```python
from build123d import *


with BuildPart() as part:
    # Sketch1 → Revolve1 (revolve)
    with BuildSketch(Plane.XY, mode=Mode.PRIVATE) as revolve1_sk:
        Polygon((0, 0), (0, 2.0095), (0.4905, 2.5), (15, 2.5), (15, 2.067), (16.5, 2.067), (16.5, 2.5), (140.5, 2.5), (140.5, 8), (145.5, 8), (145.5, 0), align=None)
    revolve(revolve1_sk.sketch.rotate(Axis((145.5, 0, 0), (-1, 0, 0)), 180), axis=Axis((145.5, 0, 0), (-1, 0, 0)))


solid = part.part
```
Input: part model. Units: mm. Frame: model coordinates. A direction names the side the tool comes from. Coordinates: 2 decimals unless noted, no trailing zeros. Write each loop counter-clockwise with the first axis right and the second up, starting at its lowest first coordinate (ties: lowest second). Pieces come first, ordered by that corner, then holes. Notation, with made-up numbers: (-40, 38) -> (5, 38) arc R32 ccw to (5, 72) -> close; hole circle Ø5 at (15, -2). An arc over 180 degrees is marked (long way). Write each question's results on one line, items separated by ' | '.
Item 1: Section query D-D on y = -5.75. Return loops of the section in (x, z).
Conclusion:
outline: (140.5, -5.56) -> (145.5, -5.56) -> (145.5, 5.56) -> (140.5, 5.56) -> close
Item 2: Mould query, pull axis X, two halves, no side actions, for faces 4 (the flat face through (145.5, 0, 0)), 5 (the cylindrical face through (15.76, -1.97, 0.62)), 6 (the flat face through (0, 0, 0)). Classes: +X half, -X half, draft (parallel to the pull), parting line (faces both ways), or undercut.
Conclusion:
face 4: +X half | face 5: undercut | face 6: -X half
Item 3: Pin query (flat end, axial travel): pin 1 Ø1 at (x, z) = (75, -2.5) entering from -Y; pin 2 Ø2 at (x, y) = (56.5, 2) entering from +Z; pin 3 Ø3 at (x, z) = (29.5, 5.5) entering from +Y; pin 4 Ø1.5 at (y, z) = (6, -5) entering from -X. Return the tip coordinate at first contact, or that it passes through.
Conclusion:
pin 1: stops at y = -1.5 | pin 2: stops at z = 2.29 | pin 3: passes through | pin 4: stops at x = 140.5
Item 4: Set-up query: faces 1 (the cylindrical face through (143.04, 1.73, -7.81)), 2 (the cylindrical face through (7.8, 2.5, 0.1)), 3 (the flat face through (15, 1, 2)). Return all of +Z, -Z, +X, -X, +Y, -Y with unobstructed straight access to the full face (end or side cutting, diameter ignored); none if empty.
Conclusion:
face 1: +X, -X | face 2: -X | face 3: none
Item 5: Material intervals for probe 1 along X at (y, z) = (-7.25, 2.25); probe 2 along Z at (x, y) = (18.5, -0.25); probe 3 along Z at (x, y) = (49, 1), sorted ascending.
Conclusion:
probe 1: x = 140.5 to 145.5 | probe 2: z = -2.49 to 2.49 | probe 3: z = -2.29 to 2.29
Item 6: Section query A-A on z = 0. Return loops of the section in (x, y), plus the area to 3 significant figures.
Conclusion:
outline: (0, -2.01) -> (0.49, -2.5) -> (15, -2.5) -> (15, -2.07) -> (16.5, -2.07) -> (16.5, -2.5) -> (140.5, -2.5) -> (140.5, -8) -> (145.5, -8) -> (145.5, 8) -> (140.5, 8) -> (140.5, 2.5) -> (16.5, 2.5) -> (16.5, 2.07) -> (15, 2.07) -> (15, 2.5) -> (0.49, 2.5) -> (0, 2.01) -> close | area: 781 mm^2
Item 7: Section query C-C on x = 46.5. Return loops of the section in (y, z).
Conclusion:
outline: circle Ø5 at (0, 0)
